Input: part model. Units: mm. Frame: model coordinates. A direction names the side the tool comes from. Coordinates: 2 decimals unless noted, no trailing zeros. Write each loop counter-clockwise with the first axis right and the second up, starting at its lowest first coordinate (ties: lowest second). Pieces come first, ordered by that corner, then holes. Notation, with made-up numbers: (18, 66.5) - (48, 66.5) arc R15 cw to (48, 84.5) - close; hole circle Ø7 at (47.25, 52.25). An arc over 180 degrees is marked (long way). Use CSV: the item, a comma, the result in double quotes.
```python
from build123d import *

# Parameters (mm, degrees)
SKETCH1_R           = 5
BOSS_EXTRUDE1_DEPTH = 300


with BuildPart() as part:
    # Sketch1 → Boss-Extrude1 (new body)
    with BuildSketch(Plane(origin=(0, 0, 0), x_dir=(1, 0, 0), z_dir=(0, 1, 0))):
        Polygon((-6, 20), (-6, 16), (-11.757359313, 16), (-5.757359313, 10), (5.757359313, 10), (11.757359313, 16), (6, 16), (6, 20), (20, 20), (20, 6), (16, 6), (16, 11.757359313), (10, 5.757359313), (10, -5.757359313), (16, -11.757359313), (16, -6), (20, -6), (20, -20), (6, -20), (6, -16), (11.757359313, -16), (5.757359313, -10), (-5.757359313, -10), (-11.757359313, -16), (-6, -16), (-6, -20), (-20, -20), (-20, -6), (-16, -6), (-16, -11.757359313), (-10, -5.757359313), (-10, 5.757359313), (-16, 11.757359313), (-16, 6), (-20, 6), (-20, 20), align=None)
        with Locations(Location((0, 0, 0), (0, 0, 270))):
            Circle(SKETCH1_R, mode=Mode.SUBTRACT)
    extrude(amount=BOSS_EXTRUDE1_DEPTH)


solid = part.part
```
(1) Reachability of faces 5 (the flat face through (13, 148, -20)), 6 (the flat face through (-10, 148, 0)), 7 (the flat face through (0, 148, -10)), 8 (the flat face through (10, 148, 0)) from +Z, -Z, +X, -X, +Y, -Y: full face, straight path, thin tool, end or side. Return the list, or none.
Check values:
face 5,"-Z, +X, -X, +Y, -Y"
face 6,"-X, +Y, -Y"
face 7,"-Z, +Y, -Y"
face 8,"+X, +Y, -Y"
(2) Ray query, probe 1 along X at (y, z) = (288, -7.5); probe 2 along X at (y, z) = (60, 0); probe 3 along X at (y, z) = (117, -17). Return the intervals inside material, ascending. Write a range as from..to.
Check values:
probe 1,"-20..-16, -11.74..11.74, 16..20"
probe 2,"-10..-5, 5..10"
probe 3,"-20..-6, 6..20"
(3) Draft query along X for faces 1 (the flat face through (8.72, 147.9, -12.96)), 2 (the flat face through (13, 148, 20)), 3 (the flat face through (-20, 148, -13)), 4 (the flat face through (-9, 148, 16)). Return one class per face: pulls with the +X half, pulls with the -X half, needs draft (parallel to the pull), parting line crosses it, or undercut.
Check values:
face 1,"undercut"
face 2,"needs draft"
face 3,"pulls with the -X half"
face 4,"undercut"
(4) Cut plane B-B on z = 0. Return loops of the section in (x, y).
Check values:
outline,"(-10, 0) - (-5, 0) - (-5, 300) - (-10, 300) - close; (5, 0) - (10, 0) - (10, 300) - (5, 300) - close"
(5) Cut plane A-A on x = 0. Return loops of the section in (y, z), and give its area (3 significant figures).
Check values:
outline,"(0, -10) - (300, -10) - (300, -5) - (0, -5) - close; (0, 5) - (300, 5) - (300, 10) - (0, 10) - close"
area,"3,000 mm^2"
(6) Pin query (flat end, axial travel): pin 1 Ø9 at (y, z) = (135, -1) entering from +X; pin 2 Ø2 at (x, y) = (2, 48.5) entering from +Z; pin 3 Ø1 at (y, z) = (137.5, 3) entering from -X. Return the tip coordinate at first contact, or that it passes through.
Check values:
pin 1,"x = 10"
pin 2,"z = 10"
pin 3,"x = -10"
